Here's how the part is built. I have some questions about the finished solid (model axes, mm). Give positions to 0.01 mm unless a question says otherwise; leave off trailing zeros. Loops run counter-clockwise (first coordinate to the right, second up) from the corner with the lowest first, then second, coordinate; pieces in that order, holes last. Notation, with made-up numbers: (37, -10.75) - (80, -10.75) arc R8 ccw to (80, 3.25) - close; hole circle Ø8 at (86, -38.5). An arc over 180 degrees is marked (long way). Use one line per item in the form item = value.
from build123d import *

# Parameters (mm, degrees)
SKETCH1_R           = 40
BOSS_EXTRUDE1_DEPTH = 20
M10_TAPPED_HOLE1_D  = 8.5
CHAMFER1_SIZE       = 70
FILLET1_R           = 20


with BuildPart() as part:
    # Sketch1 → Boss-Extrude1 (new body)
    with BuildSketch(Plane.XY):
        with BuildLine():
            Line((0, -70), (0, 70))
            Line((0, 70), (-100.453845954, 103.30202446))
            ThreePointArc((-100.453845954, 103.30202446), (-144.970416858, 163.039149842), (-104.13740045, 225.352182227))
            Line((-104.13740045, 225.352182227), (20, 275))
            Line((20, 275), (370, 275))
            Line((370, 275), (370, -275))
            Line((370, -275), (20, -275))
            Line((20, -275), (-104.13740045, -225.352182227))
            ThreePointArc((-104.13740045, -225.352182227), (-144.970416858, -163.039149842), (-100.453845954, -103.30202446))
            Line((-100.453845954, -103.30202446), (0, -70))
        make_face()
        with Locations((-80, 165)):
            Circle(SKETCH1_R, mode=Mode.SUBTRACT)
        with Locations(Location((-80, -165, 0), (0, 0, 180))):
            Circle(SKETCH1_R, mode=Mode.SUBTRACT)
        Polygon((231, 158.5), (231, 114.5), (30, 114.5), (30, 215.5), (231, 215.5), (231, 171.5), (331, 171.5), (331, 158.5), align=None, mode=Mode.SUBTRACT)
        Polygon((331, -171.5), (331, -158.5), (231, -158.5), (231, -114.5), (30, -114.5), (30, -215.5), (231, -215.5), (231, -171.5), align=None, mode=Mode.SUBTRACT)
    extrude(amount=BOSS_EXTRUDE1_DEPTH)

    # M10 Tapped Hole1 (through all)
    with Locations(Plane.XY.offset(20)):
        with Locations((-8, 195), (-8, 135), (-8, -135), (-8, -195)):
            Hole(M10_TAPPED_HOLE1_D / 2)

    # Chamfer1
    chamfer1_edges = [part.edges().sort_by_distance(p)[0] for p in [
        (370, 275, 10),
        (370, -275, 10),
    ]]
    chamfer(chamfer1_edges, length=CHAMFER1_SIZE)

    # Fillet1
    fillet1_edges = [part.edges().sort_by_distance(p)[0] for p in [
        (0, -70, 10),
        (0, 70, 10),
    ]]
    fillet(fillet1_edges, radius=FILLET1_R)


solid = part.part
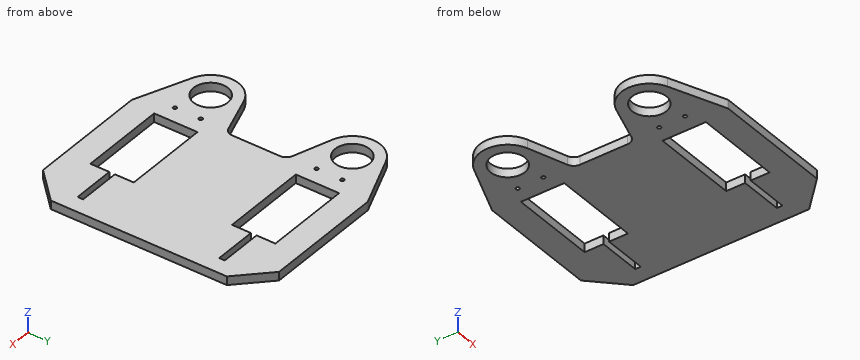
(1) If I drill on probe 1 along Y at (x, z) = (115.5, 18.75); probe 2 along X at (y, z) = (-165, 15); probe 3 along Y at (x, z) = (279.5, 17.5), over which ranges is the centre line in solid material (lowest first)?
Geometry says:
probe_1 = -275 to -215.5, -114.5 to 114.5, 215.5 to 275
probe_2 = -145 to -120, -40 to 30, 331 to 370
probe_3 = -275 to -171.5, -158.5 to 158.5, 171.5 to 275
(2) For P1, Ø6, axis at y = 197, z = 5, coming from the -X side; P2, Ø1, axis at y = 10, z = 3, coming from the -X side; P3, Ø6, axis at y = 204, z = 3.5, coming from the -X side, each with a flat end and sliding along its axis, tell me the tip position at first contact or that it passes through.
Geometry says:
P1 = -138.17
P2 = 0
P3 = -134.12
(3) If we section it at A-A (y = -165): List the corners of the cut face in (x, z) for me.
Geometry says:
outline = (-145, 0) - (-120, 0) - (-120, 20) - (-145, 20) - close; (-40, 0) - (30, 0) - (30, 20) - (-40, 20) - close; (331, 0) - (370, 0) - (370, 20) - (331, 20) - close
(4) If we section it at C-C (x = -82): List the corners of the cut face in (y, z) for me.
Geometry says:
outline = (-234.21, 0) - (-204.95, 0) - (-204.95, 20) - (-234.21, 20) - close; (-125.05, 0) - (-97.18, 0) - (-97.18, 20) - (-125.05, 20) - close; (97.18, 0) - (125.05, 0) - (125.05, 20) - (97.18, 20) - close; (204.95, 0) - (234.21, 0) - (234.21, 20) - (204.95, 20) - close
(5) If we section it at B-B (x = 286.5): List the corners of the cut face in (y, z) for me.
Geometry says:
outline = (-275, 0) - (-171.5, 0) - (-171.5, 20) - (-275, 20) - close; (-158.5, 0) - (158.5, 0) - (158.5, 20) - (-158.5, 20) - close; (171.5, 0) - (275, 0) - (275, 20) - (171.5, 20) - close
(6) If we section it at D-D (z = 16): Give the number of separate pieces and of enclosed holes in the cut face, plus the area to 3 significant figures.
Geometry says:
separate_pieces = 1
enclosed_holes = 8
area = 185,000 mm²
